Answer from the drawing. Dimensions are ordinates in mm from the lowest x, y and z of the part. A direction names the side the tool comes from. Coordinates: 2 decimals unless noted, no trailing zeros. Write each loop counter-clockwise with the first axis right and the second up, starting at its lowest first coordinate (ties: lowest second). Pieces come first, ordered by that corner, then holes. Notation, with made-up numbers: (21.5, 72.5) - (58.5, 72.5) arc R20 ccw to (58.5, 84.5) - close; hole circle Ø9 at (81.5, 57). An arc over 180 degrees is marked (long way). Use one line per item in the form item = value. Start each with the question number.
Item 1: Consider probe 1 along Y at (x, z) = (0.4, 1.5); probe 2 along X at (y, z) = (4.6, 2.8); probe 3 along X at (y, z) = (5.6, 1.7). Determine where each line is inside the solid, lowest interval first.
Item 2: A cutting plane is placed at C-C (y = 2.9). Write down the section's boundary in (x, z).
Item 3: For the marked faces 1 and 2, determine the directions among +Z, -Z, +X, -X, +Y, -Y from which every point of the face is accessible in a straight line to the end or side of a thin tool.
Item 4: A cutting plane is placed at A-A (z = 2). Write down the section's boundary in (x, y).
Item 5: A cutting plane is placed at B-B (x = 2). Write down the section's boundary in (y, z), then the cut area to 3 significant figures.
Item 6: A cutting plane is placed at D-D (y = 3.55). Write down the section's boundary in (x, z).
Item 7: Given pin 1 (2 mm diameter, centred on y = 4.5, z = 0.5, fed in from -X), flat-ended and moving along its own axis, determine where the tip first touches the part or whether it passes through.
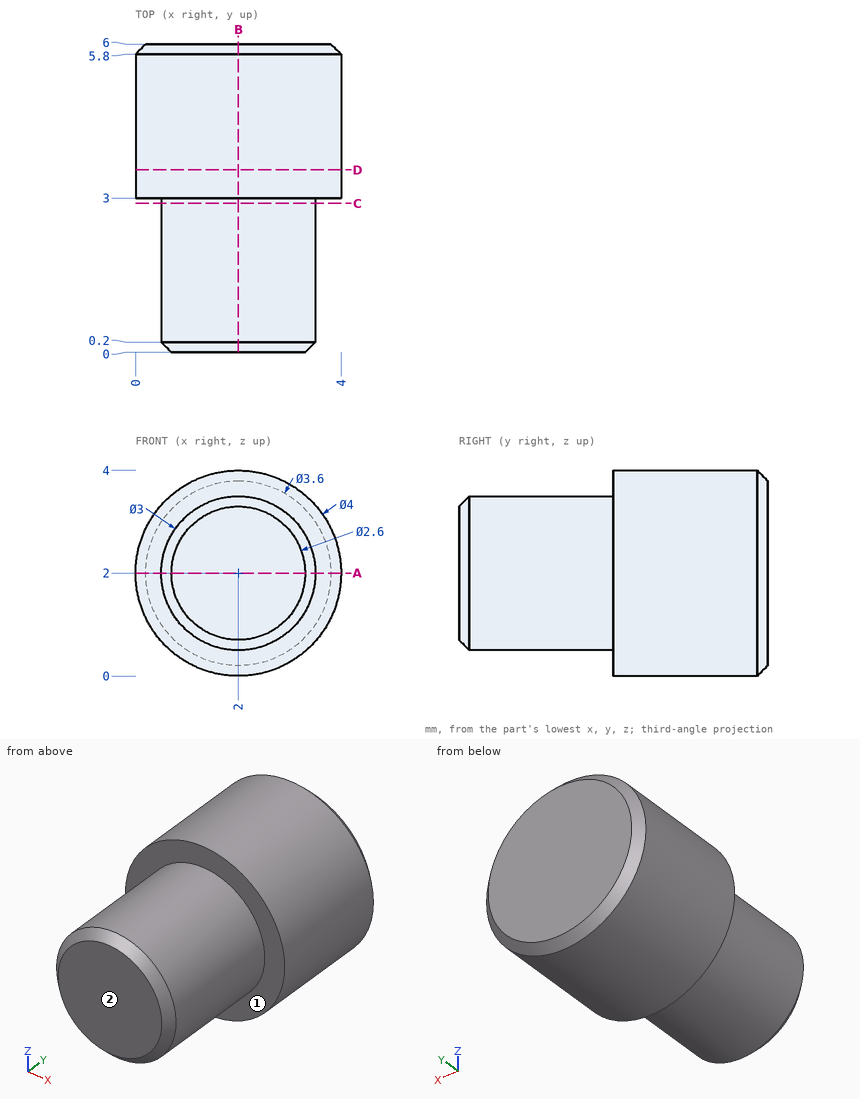
Answer:
q1.probe_1 = 3 to 6
q1.probe_2 = 0.17 to 3.83
q1.probe_3 = 0.02 to 3.98
q2.outline = circle Ø3 at (2, 2)
q3.face_1 = -Y
q3.face_2 = +Z, -Z, +X, -X, -Y
q4.outline = (0, 3) - (0.5, 3) - (0.5, 0.2) - (0.7, 0) - (3.3, 0) - (3.5, 0.2) - (3.5, 3) - (4, 3) - (4, 5.8) - (3.8, 6) - (0.2, 6) - (0, 5.8) - close
q5.outline = (0, 0.7) - (0.2, 0.5) - (3, 0.5) - (3, 0) - (5.8, 0) - (6, 0.2) - (6, 3.8) - (5.8, 4) - (3, 4) - (3, 3.5) - (0.2, 3.5) - (0, 3.3) - close
q5.area = 20.9 mm²
q6.outline = circle Ø4 at (2, 2)
q7.pin_1 = 0.06
